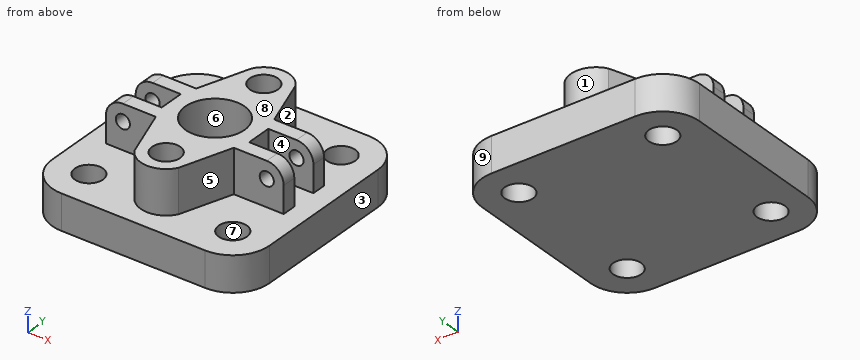
from build123d import *

# Parameters (mm, degrees)
BASE_PLATE_DEPTH         = 25
FLANGE_BOSS_DEPTH        = 31
LUG_SLOT_1_DEPTH         = 50
LUG_SLOT_2_DEPTH         = 50
LUG_PIN_HOLES_SKETCH_R   = 5
LUG_PIN_HOLES_2X_DEPTH   = 50
FLANGE_HOLES_SKETCH_R    = 10
FLANGE_HOLES_2X_DEPTH    = 22
CENTRE_BORE_SKETCH_R     = 21
CENTRE_BORE_42_DEPTH     = 42
CORNER_HOLES_SKETCH_R    = 10
CORNER_HOLES_4X_20_DEPTH = 42


with BuildPart() as part:
    # Base Plate Sketch → Base Plate (new body)
    with BuildSketch(Plane.XY):
        with BuildLine():
            Line((0, -26), (0, -128))
            ThreePointArc((0, -128), (7.615223689, -146.384776311), (26, -154))
            Line((26, -154), (128, -154))
            ThreePointArc((128, -154), (146.384776311, -146.384776311), (154, -128))
            Line((154, -128), (154, -26))
            ThreePointArc((154, -26), (146.384776311, -7.615223689), (128, 0))
            Line((128, 0), (26, 0))
            ThreePointArc((26, 0), (7.615223689, -7.615223689), (0, -26))
        make_face()
    extrude(amount=BASE_PLATE_DEPTH)

    # Flange Boss Sketch → Flange Boss (add)
    with BuildSketch(Plane.XY.offset(25)):
        with BuildLine():
            Line((14, -96), (49.353610872, -96))
            Line((49.353610872, -96), (61.447265664, -132.061592281))
            ThreePointArc((61.447265664, -132.061592281), (77, -141), (92.552734336, -132.061592281))
            Line((92.552734336, -132.061592281), (104.646389128, -96))
            Line((104.646389128, -96), (140, -96))
            Line((140, -96), (140, -86))
            Line((140, -86), (108, -86))
            Line((108, -86), (108, -68))
            Line((108, -68), (140, -68))
            Line((140, -68), (140, -58))
            Line((140, -58), (104.646389128, -58))
            Line((104.646389128, -58), (92.552734336, -21.938407719))
            ThreePointArc((92.552734336, -21.938407719), (77, -13), (61.447265664, -21.938407719))
            Line((61.447265664, -21.938407719), (49.353610872, -58))
            Line((49.353610872, -58), (14, -58))
            Line((14, -58), (14, -68))
            Line((14, -68), (46, -68))
            Line((46, -68), (46, -77))
            Line((46, -77), (46, -86))
            Line((46, -86), (14, -86))
            Line((14, -86), (14, -96))
        make_face()
    extrude(amount=FLANGE_BOSS_DEPTH)

    # Lug Slot 1 Sketch → Lug Slot 1 (cut)
    with BuildSketch(Plane.XZ.offset(96)):
        with BuildLine():
            Line((140, 56), (140, 44))
            ThreePointArc((140, 44), (136.485281374, 52.485281374), (128, 56))
            Line((128, 56), (140, 56))
        make_face()
    extrude(amount=-LUG_SLOT_1_DEPTH, mode=Mode.SUBTRACT)

    # Lug Slot 2 Sketch → Lug Slot 2 (cut)
    with BuildSketch(Plane.XZ.offset(96)):
        with BuildLine():
            Line((14, 56), (26, 56))
            ThreePointArc((26, 56), (17.514718626, 52.485281374), (14, 44))
            Line((14, 44), (14, 56))
        make_face()
    extrude(amount=-LUG_SLOT_2_DEPTH, mode=Mode.SUBTRACT)

    # Lug Pin Holes Sketch → Lug Pin Holes 2x (cut)
    with BuildSketch(Plane.XZ.offset(96)):
        with Locations(Location((128, 44, 0), (0, 0, 270))):
            Circle(LUG_PIN_HOLES_SKETCH_R)
        with Locations(Location((26, 44, 0), (0, 0, 270))):
            Circle(LUG_PIN_HOLES_SKETCH_R)
    extrude(amount=-LUG_PIN_HOLES_2X_DEPTH, mode=Mode.SUBTRACT)

    # Flange Holes Sketch → Flange Holes 2x (cut)
    with BuildSketch(Plane.XY.offset(56)):
        with Locations((77, -31)):
            Circle(FLANGE_HOLES_SKETCH_R)
        with Locations((77, -123)):
            Circle(FLANGE_HOLES_SKETCH_R)
    extrude(amount=-FLANGE_HOLES_2X_DEPTH, mode=Mode.SUBTRACT)

    # Centre Bore Sketch → Centre Bore Ø42 (cut)
    with BuildSketch(Plane.XY.offset(56)):
        with Locations((77, -77)):
            Circle(CENTRE_BORE_SKETCH_R)
    extrude(amount=-CENTRE_BORE_42_DEPTH, mode=Mode.SUBTRACT)

    # Corner Holes Sketch → Corner Holes 4xØ20 (cut)
    with BuildSketch(Plane.XY.offset(25)):
        with Locations((26, -26)):
            Circle(CORNER_HOLES_SKETCH_R)
        with Locations((128, -26)):
            Circle(CORNER_HOLES_SKETCH_R)
        with Locations((128, -128)):
            Circle(CORNER_HOLES_SKETCH_R)
        with Locations((26, -128)):
            Circle(CORNER_HOLES_SKETCH_R)
    extrude(amount=-CORNER_HOLES_4X_20_DEPTH, mode=Mode.SUBTRACT)


solid = part.part
Model file for the job. Use its own axes, mm. Face numbers are marked on the shaded views. A direction names the side the tool comes from. Give positions to 0.01 mm unless a question says otherwise; leave off trailing zeros. Loops run counter-clockwise (first coordinate to the right, second up) from the corner with the lowest first, then second, coordinate; pieces in that order, holes last. Notation, with made-up numbers: (33.5, 25.5) -> (61.5, 25.5) arc R22 cw to (61.5, 49.5) -> close; hole circle Ø6 at (52.5, 47.25). An arc over 180 degrees is marked (long way). Use a Markdown table: item, result. Add a question column.
(1) Tool access for the marked faces 1, 2, 3, 4 and 5: list every direction of +Z, -Z, +X, -X, +Y, -Y with a clear straight run to the whole face (end or side of a thin tool).
(2) Slice it at D-D on x = 18. List the corners of the cut face in (y, z).
(3) Slice it at A-A on z = 18. List the corners of the cut face in (x, y), and give its area (3 significant figures).
(4) Slice it at B-B on x = 77. List the corners of the cut face in (y, z).
(5) Slice it at C-C on z = 9. List the corners of the cut face in (x, y).
(6) Wall check: line 1 along Y through (x, z) = (128, 16); line 2 along Y through (x, z) = (117, 34.5); line 3 along Y through (x, z) = (76, 16.5). Give the ranges that are in metal, low to high.
(7) Mould opens along X. For the marked faces 6, 7, 8 and 9 say: +X half, -X half, draft (parallel to the pull), parting line (faces both ways), or undercut.
(8) Drop flat-ended pins along their axis: pin 1 Ø1.5 at (y, z) = (-26.5, 44.5) entering from +X; pin 2 Ø10 at (y, z) = (-124, 49.5) entering from -X; pin 3 Ø12.5 at (x, y) = (80.5, -86.5) entering from +Z; pin 4 Ø6 at (x, z) = (128, 44) entering from +Y. Give the stop position or say it passes through.
Filled sheet:
| question | item | result |
|---|---|---|
| 1 | face 1 | +Z, +Y |
| 1 | face 2 | +Z, +X, +Y |
| 1 | face 3 | +Z, -Z, +X, +Y, -Y |
| 1 | face 4 | +Z, +X |
| 1 | face 5 | +Z, +X, -Y |
| 2 | outline | (-152.74, 0) -> (-134, 0) -> (-134, 25) -> (-152.74, 25) -> close; (-122, 0) -> (-32, 0) -> (-32, 25) -> (-58, 25) -> (-58, 52.94) -> (-68, 52.94) -> (-68, 25) -> (-86, 25) -> (-86, 52.94) -> (-96, 52.94) -> (-96, 25) -> (-122, 25) -> close; (-20, 0) -> (-1.26, 0) -> (-1.26, 25) -> (-20, 25) -> close |
| 3 | outline | (0, -128) arc R26 ccw to (26, -154) -> (128, -154) arc R26 ccw to (154, -128) -> (154, -26) arc R26 ccw to (128, 0) -> (26, 0) arc R26 ccw to (0, -26) -> close; hole circle Ø20 at (26, -128); hole circle Ø20 at (26, -26); hole circle Ø42 at (77, -77); hole circle Ø20 at (128, -128); hole circle Ø20 at (128, -26) |
| 3 | area | 20,500 mm2 |
| 4 | outline | (-154, 0) -> (0, 0) -> (0, 25) -> (-13, 25) -> (-13, 56) -> (-21, 56) -> (-21, 34) -> (-41, 34) -> (-41, 56) -> (-56, 56) -> (-56, 14) -> (-98, 14) -> (-98, 56) -> (-113, 56) -> (-113, 34) -> (-133, 34) -> (-133, 56) -> (-141, 56) -> (-141, 25) -> (-154, 25) -> close |
| 5 | outline | (0, -128) arc R26 ccw to (26, -154) -> (128, -154) arc R26 ccw to (154, -128) -> (154, -26) arc R26 ccw to (128, 0) -> (26, 0) arc R26 ccw to (0, -26) -> close; hole circle Ø20 at (26, -128); hole circle Ø20 at (26, -26); hole circle Ø20 at (128, -128); hole circle Ø20 at (128, -26) |
| 6 | line 1 | -154 to -138, -118 to -36, -16 to 0 |
| 6 | line 2 | -96 to -86, -68 to -58 |
| 6 | line 3 | -154 to -97.98, -56.02 to 0 |
| 7 | face 6 | undercut |
| 7 | face 7 | undercut |
| 7 | face 8 | draft |
| 7 | face 9 | +X half |
| 8 | pin 1 | x = 94.33 |
| 8 | pin 2 | x = 57.07 |
| 8 | pin 3 | z = 14 |
| 8 | pin 4 | through |
